```python
from build123d import *

# Parameters (mm, degrees)
SKETCH2_R           = 1
BOSS_EXTRUDE1_DEPTH = 5
CHAMFER1_SIZE       = 0.5


with BuildPart() as part:
    # Sketch1 → Revolve1 (revolve)
    with BuildSketch(Plane.XY, mode=Mode.PRIVATE) as revolve1_sk:
        with BuildLine():
            Line((0, 0), (0, 2))
            Line((0, 2), (16.22853262, 2))
            ThreePointArc((16.22853262, 2), (16.998410661, 1.975278193), (17.765116572, 1.901214634))
            Line((17.765116572, 1.901214634), (24.040853529, 1.090944675))
            ThreePointArc((24.040853529, 1.090944675), (24.726117087, 0.72631299), (25, 0))
            Line((25, 0), (0, 0))
        make_face()
    revolve(revolve1_sk.sketch.rotate(Axis((0, 0, 0), (1, 0, 0)), 90), axis=Axis((0, 0, 0), (1, 0, 0)))

    # Sketch2 → Boss-Extrude1 (add)
    with BuildSketch(Plane.ZY):
        Circle(SKETCH2_R)
    extrude(amount=BOSS_EXTRUDE1_DEPTH)

    # Chamfer1
    chamfer1_edges = [part.edges().sort_by_distance(p)[0] for p in [
        (-5, 0, -1),
    ]]
    chamfer(chamfer1_edges, length=CHAMFER1_SIZE)


solid = part.part
```
Read the model definition and answer for the solid it produces. Units are mm, in the model's axes. A direction names the side the tool comes from. Give positions to 0.01 mm unless a question says otherwise; leave off trailing zeros. Loops run counter-clockwise (first coordinate to the right, second up) from the corner with the lowest first, then second, coordinate; pieces in that order, holes last.
Item 1: Find the intervals of material crossed by line 1 along Y through (x, z) = (21.5, -0.9); line 2 along Z through (x, y) = (15.75, 0.95); line 3 along Z through (x, y) = (23.5, 0.05), in increasing order.
Item 2: Each of these flat-tipped pins is pushed along its axis until it touches: pin 1 Ø2 at (x, z) = (20, 1) entering from +Y; pin 2 Ø1 at (y, z) = (-1, 1.5) entering from -X; pin 3 Ø1 at (x, z) = (14.5, 1) entering from -Y. Where does it stop, or does it pass through?
Item 3: The part is cut by section A-A (x = 4). Write down the section's boundary in (y, z).
Item 4: For faces 1 (the flat face through (-5, 0, 0)), 2 (the flat face through (0, 1, -1)), determine the directions among +Z, -Z, +X, -X, +Y, -Y from which every point of the face is accessible in a straight line to the end or side of a thin tool.
Item 5: The part is cut by section B-B (x = 19.75). Write down the section's boundary in (y, z), and give its area (3 significant figures).
Taken from the geometry:
1. line 1: y = -1.1 to 1.1
1. line 2: z = -1.76 to 1.76
1. line 3: z = -1.16 to 1.16
2. pin 1: stops at y = 1.68
2. pin 2: stops at x = 0
2. pin 3: stops at y = -1.94
3. outline: circle Ø4 at (0, 0)
4. face 1: +Z, -Z, -X, +Y, -Y
4. face 2: -X
5. outline: circle Ø3.29 at (0, 0)
5. area: 8.50 mm2
